Source: CAD feature listing. Evaluate the final solid. Frame: model axes, mm. A direction names the side the tool comes from. Give positions to 0.01 mm unless a question says otherwise; leave off trailing zeros. Order: outer loops, then holes, each group sorted by start corner. A loop starts at its lowest first (then second) coordinate and runs counter-clockwise, first axis right, second up. Notation, with made-up numbers: (57.5, -25) -> (107.5, -25) arc R28 cw to (107.5, -4) -> close; hole circle Ø2 at (-28.5, 1). An arc over 180 degrees is marked (long way). Use CSV: the item, a comma, the result in double quotes.
```python
from build123d import *

# Parameters (mm, degrees)
SKETCH_1_R                    = 70
SKETCH_1_R_2                  = 21.5
EXTRUDE_1_DEPTH               = 40
HOLE_WIZARD_M16_1_D           = 14
HOLE_WIZARD_M16_1_DEPTH       = 27.793975667
HOLE_WIZARD_M16_1_CSINK_D     = 16.05
HOLE_WIZARD_M16_1_CSINK_ANGLE = 90
HOLE_WIZARD_M16_1_TIP         = 4.206024333
HOLE_WIZARD_M16_3_D           = 14
HOLE_WIZARD_M16_3_DEPTH       = 27.793975667
HOLE_WIZARD_M16_3_CSINK_D     = 16.05
HOLE_WIZARD_M16_3_CSINK_ANGLE = 90
HOLE_WIZARD_M16_3_TIP         = 4.206024333


with BuildPart() as part:
    # 草图1 → 凸台-拉伸1 (new body)
    with BuildSketch(Plane(origin=(0, 0, 0), x_dir=(1, 0, 0), z_dir=(0, 1, 0))):
        with Locations(Location((0, 0, 0), (0, 0, 270))):
            Circle(SKETCH_1_R)
        with Locations(Location((0, 0, 0), (0, 0, 270))):
            Circle(SKETCH_1_R_2, mode=Mode.SUBTRACT)
    extrude(amount=EXTRUDE_1_DEPTH)

    # M16 螺纹孔1
    with Locations(Plane(origin=(0, 40, 0), x_dir=(1, 0, 0), z_dir=(0, 1, 0))):
        with Locations((0, 50), (50, 0), (0, -50), (-50, 0)):
            CounterSinkHole(HOLE_WIZARD_M16_1_D / 2, HOLE_WIZARD_M16_1_CSINK_D / 2, depth=HOLE_WIZARD_M16_1_DEPTH, counter_sink_angle=HOLE_WIZARD_M16_1_CSINK_ANGLE)
            with Locations((0, 0, -(HOLE_WIZARD_M16_1_DEPTH + HOLE_WIZARD_M16_1_TIP / 2))):  # 118° drill point
                Cone(0, HOLE_WIZARD_M16_1_D / 2, HOLE_WIZARD_M16_1_TIP, mode=Mode.SUBTRACT)

    # M16 螺纹孔3
    with Locations(Plane(origin=(0, 0, 0), x_dir=(-1, 0, 0), z_dir=(0, -1, 0))):
        with Locations((-35.355339059, 35.355339059), (35.355339059, 35.355339059), (35.355339059, -35.355339059), (-35.355339059, -35.355339059)):
            CounterSinkHole(HOLE_WIZARD_M16_3_D / 2, HOLE_WIZARD_M16_3_CSINK_D / 2, depth=HOLE_WIZARD_M16_3_DEPTH, counter_sink_angle=HOLE_WIZARD_M16_3_CSINK_ANGLE)
            with Locations((0, 0, -(HOLE_WIZARD_M16_3_DEPTH + HOLE_WIZARD_M16_3_TIP / 2))):  # 118° drill point
                Cone(0, HOLE_WIZARD_M16_3_D / 2, HOLE_WIZARD_M16_3_TIP, mode=Mode.SUBTRACT)


solid = part.part
```
1. Section query B-B on z = -18. Return loops of the section in (x, y), plus the area to 3 significant figures.
Answer below:
outline,"(-67.65, 0) -> (-11.76, 0) -> (-11.76, 40) -> (-67.65, 40) -> close; (11.76, 0) -> (67.65, 0) -> (67.65, 40) -> (11.76, 40) -> close"
area,"4,470 mm²"
2. Mould query, pull axis X, two halves, no side actions, for faces 4 (the cylindrical face through (34.444, 14.597, 28.415)), 5 (the flat face through (-15, 40, -17)). Classes: released by +X, released by -X, zero draft, split by the parting line, or undercut.
Answer below:
face 4,"undercut"
face 5,"zero draft"
3. Access query for faces 1 (the cylindrical face through (43.323, 25.403, -2.103)), 2 (the cylindrical face through (33.84, 14.6, -28.52)), 3 (the flat face through (-15, 0, -17)). Directions: +Z, -Z, +X, -X, +Y, -Y. A direction counts if a zero-diameter tool reaches every point of the face in a straight line with its end or side. Return the directions, or none.
Answer below:
face 1,"+Y"
face 2,"-Y"
face 3,"+Z, -Z, +X, -X, -Y"
4. Section query C-C on y = 4. Return loops of the section in (x, z).
Answer below:
outline,"circle Ø140 at (0, 0); hole circle Ø14 at (-35.36, -35.36); hole circle Ø14 at (-35.36, 35.36); hole circle Ø43 at (0, 0); hole circle Ø14 at (35.36, -35.36); hole circle Ø14 at (35.36, 35.36)"
5. Section query A-A on y = 15.5. Count the separate pieces of the cut face and the enclosed holes in it, plus the area to 3 significant figures.
Answer below:
separate pieces,"1"
enclosed holes,"9"
area,"12,700 mm²"
6. Ray query, line 1 along X through (y, z) = (11, -30); line 2 along Z through (x, y) = (-29, 15); line 3 along X through (y, z) = (14, -8). Return the intervals inside material, ascending.
Answer below:
line 1,"x = -63.25 to -39.86, -30.85 to 30.85, 39.86 to 63.25"
line 2,"z = -63.71 to -38.29, -32.42 to 32.42, 38.29 to 63.71"
line 3,"x = -69.54 to -19.96, 19.96 to 69.54"
7. Pin query (flat end, axial travel): P1, Ø12, axis at x = -7, y = 21, coming from the +Z side; P2, Ø12.5, axis at x = -35.36, z = 35.36, coming from the -Y side; P3, Ø12.5, axis at x = 50, z = 0, coming from the +Y side; P4, Ø18, axis at x = 0, z = -50, coming from the +Y side. Return the tip coordinate at first contact, or that it passes through.
Answer below:
P1,"stops at z = 69.99"
P2,"stops at y = 28.24"
P3,"stops at y = 11.76"
P4,"stops at y = 40"
